The listing builds one solid part. Answer for the finished solid, in the listing's coordinates (mm). A direction names the side the tool comes from. Give positions to 0.01 mm unless a question says otherwise; leave off trailing zeros. Loops run counter-clockwise (first coordinate to the right, second up) from the corner with the lowest first, then second, coordinate; pieces in that order, holes last. Notation, with made-up numbers: M -1,58 L 39,58 A11 cw 39,77 Z; hole C 0.25,-25.5 d1. An arc over 180 degrees is marked long. Use one line per item in the form item = value. Start each with the question number.
1. The part is cut by section B-B (y = 36.5). Write down the section's boundary in (x, z).
2. The part is cut by section C-C (x = 7.75). Write down the section's boundary in (y, z).
3. The part is cut by section A-A (z = -21). Write down the section's boundary in (x, y), and give its area (3 significant figures).
4. The part is cut by section D-D (y = 24). Write down the section's boundary in (x, z), and give its area (3 significant figures).
5. The mould has two halves that part along Y. Classify faces 6 (the face through (7.042, 35.391, -31.577)), 7 (the face through (7, 29, -36)), 8 (the face through (7.448, 17.521, -30.655)), 9 (the face through (6, 13, -14)): released by +Y, released by -Y, zero draft, split by the parting line, or undercut.
6. For faces 1 (the face through (4.54, 6.29, 7.55)), 2 (the face through (5, 7, 0)), 3 (the face through (5, 45, 1)), 4 (the face through (4, 29, -25)), 5 (the face through (7.042, 36.021, -22.155)), determine the directions among +Z, -Z, +X, -X, +Y, -Y from which every point of the face is accessible in a straight line to the end or side of a thin tool.
7. Straight lines are drawn through the part: line 1 (Z direction, x = 5, y = 4.25); line 2 (Z direction, x = 6.75, y = 12); line 3 (Z direction, x = 1.5, y = 11.5). For each, find the intervals that lie inside material, in ascending order. Write a range as from..to.
8. Each of these flat-tipped pins is pushed along its axis until it touches: pin 1 Ø5 at (y, z) = (17, -7) entering from +X; pin 2 Ø5 at (x, y) = (2.5, 5) entering from -Z; pin 3 Ø3.5 at (x, z) = (5, 5.5) entering from -Y. Where does it stop, or does it pass through?
from build123d import *

# Parameters (mm, degrees)
EXTRUDE_THIN1_DEPTH   = 25
SKETCH2_W             = 36
SKETCH2_H             = 32
BOSS_EXTRUDE1_DEPTH   = 10
SKETCH5_W             = 4
SKETCH5_H             = 22
CUT_EXTRUDE1_DEPTH    = 68.424031324
SKETCH6_W             = 55.512258346
SKETCH6_H             = 44.910131752
CUT_EXTRUDE2_DEPTH    = 10
M5_TAPPED_HOLE1_D     = 4.2
M5_TAPPED_HOLE1_DEPTH = 12.4
M5_TAPPED_HOLE1_TIP   = 1.2618073
M3_TAPPED_HOLE1_D     = 2.5
SKETCH11_W            = 4.8
SKETCH11_H            = 4
BOSS_EXTRUDE2_DEPTH   = 0.8
M3_TAPPED_HOLE2_D     = 2.5


with BuildPart() as part:
    # Sketch1 → Extrude-Thin1 (new body)
    with BuildSketch(Plane.XY):
        Polygon((-15, 0), (0, 0), (0, 45), (10, 45), (10, -10), (-15, -10), align=None)
    extrude(amount=EXTRUDE_THIN1_DEPTH)

    # Sketch2 → Boss-Extrude1 (add)
    with BuildSketch(Plane.ZY):
        with Locations((-18, 29)):
            Rectangle(SKETCH2_W, SKETCH2_H)
    extrude(amount=-BOSS_EXTRUDE1_DEPTH)

    # Sketch5 → Cut-Extrude1 (cut, through all)
    with BuildSketch(Plane(origin=(0, 45, 0), x_dir=(1, 0, 0), z_dir=(0, 1, 0))):
        with Locations((2, 25)):
            Rectangle(SKETCH5_W, SKETCH5_H)
    extrude(amount=-CUT_EXTRUDE1_DEPTH, mode=Mode.SUBTRACT)

    # Sketch6 → Cut-Extrude2 (cut)
    with BuildSketch(Plane.XZ.offset(10)):
        with Locations((-2.5, 9.73543964)):
            Rectangle(SKETCH6_W, SKETCH6_H)
    extrude(amount=-CUT_EXTRUDE2_DEPTH, mode=Mode.SUBTRACT)

    # M5 Tapped Hole1
    with Locations(Plane(origin=(0, 0, 0), x_dir=(-1, 0, 0), z_dir=(0, -1, 0))):
        with Locations((-5, -5.5), (-5, -19.5)):
            Hole(M5_TAPPED_HOLE1_D / 2, depth=M5_TAPPED_HOLE1_DEPTH)
            with Locations((0, 0, -(M5_TAPPED_HOLE1_DEPTH + M5_TAPPED_HOLE1_TIP / 2))):  # 118° drill point
                Cone(0, M5_TAPPED_HOLE1_D / 2, M5_TAPPED_HOLE1_TIP, mode=Mode.SUBTRACT)

    # M3 Tapped Hole1 (through all)
    with Locations(Plane.ZY.offset(-4)):
        with Locations((-31, 36.5), (-21, 36.5)):
            Hole(M3_TAPPED_HOLE1_D / 2)

    # Sketch11 → Boss-Extrude2 (add)
    with BuildSketch(Plane(origin=(10, 0, 0), x_dir=(0, 0, -1), z_dir=(1, 0, 0))):
        with Locations((29.5, 18)):
            Rectangle(SKETCH11_W, SKETCH11_H)
    extrude(amount=BOSS_EXTRUDE2_DEPTH)

    # M3 Tapped Hole2 (through all)
    with Locations(Plane.ZY):
        with Locations((-29.5, 18)):
            Hole(M3_TAPPED_HOLE2_D / 2)


solid = part.part
Derived:
q1.outline = M 0,-14 L 4,-14 L 4,-19.75 L 10,-19.75 L 10,25 L 0,25 Z; M 4,-36 L 10,-36 L 10,-32.25 L 4,-32.25 Z; M 4,-29.75 L 10,-29.75 L 10,-22.25 L 4,-22.25 Z
q2.outline = M 0,0 L 13,0 L 13,-36 L 45,-36 L 45,25 L 0,25 Z; hole C 18,-29.5 d2.5; hole C 36.5,-31 d2.5; hole C 36.5,-21 d2.5
q3.outline = M 4,13 L 10,13 L 10,35.25 L 4,35.25 Z; M 4,37.75 L 10,37.75 L 10,45 L 4,45 Z
q3.area = 177 mm2
q4.outline = M 0,-14 L 4,-14 L 4,-36 L 10,-36 L 10,25 L 0,25 Z
q4.area = 522 mm2
q5.face_6 = undercut
q5.face_7 = zero draft
q5.face_8 = undercut
q5.face_9 = released by -Y
q6.face_1 = -Y
q6.face_2 = -Z, +X, -X, -Y
q6.face_3 = +Z, -Z, +X, -X, +Y
q6.face_4 = -Z, -X, +Y, -Y
q6.face_5 = +X, -X
q7.line_1 = 0..3.4, 7.6..17.4, 21.6..25
q7.line_2 = 0..4.34, 6.66..18.34, 20.66..25
q7.line_3 = 0..25
q8.pin_1 = 10
q8.pin_2 = 0
q8.pin_3 = 12.61
